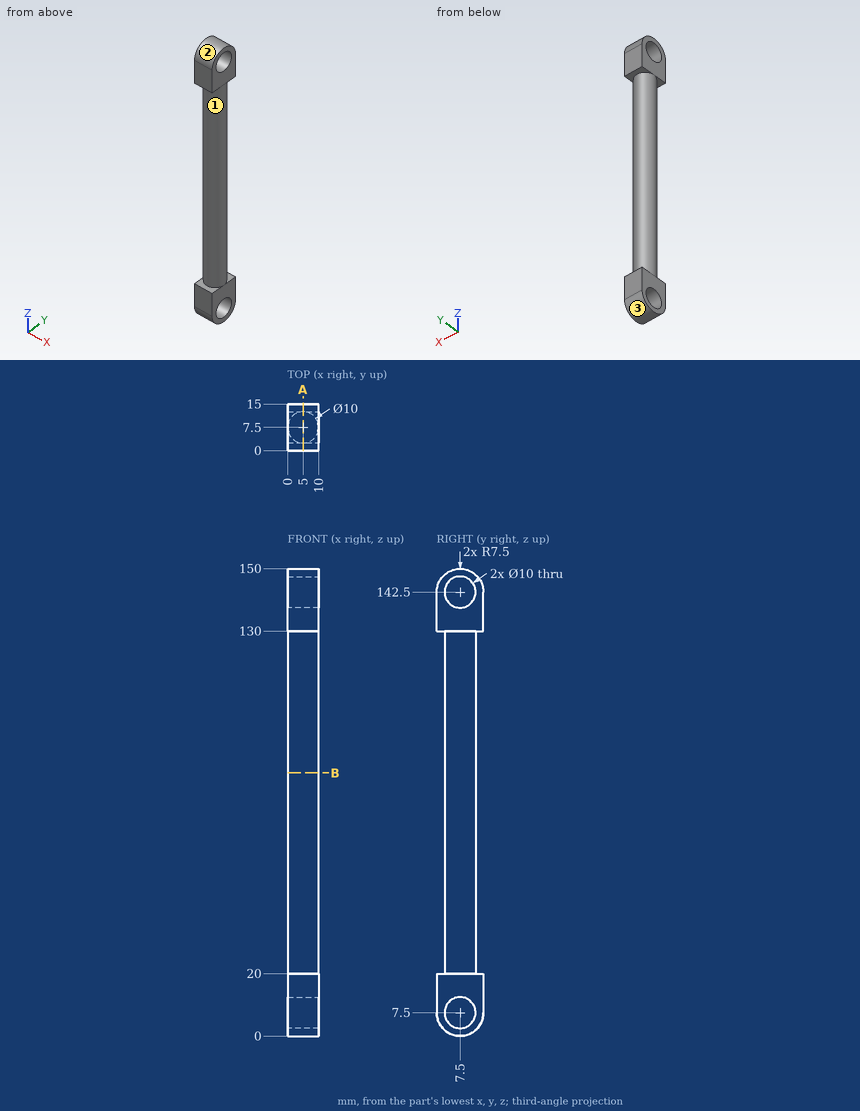
Design review of the part shown in the three views and the two pictorial views. Dimensions are in mm from the part's minimum x, y and z. Coordinates: 2 decimals unless noted, no trailing zeros. Order: outer loops, then holes, each group sorted by start corner. A loop starts at its lowest first (then second) coordinate and runs counter-clockwise, first axis right, second up. Notation, with made-up numbers: (53, 53.5) - (98, 53.5) arc R25 cw to (98, 66.5) - close; hole circle Ø6 at (60.25, 12). An arc over 180 degrees is marked (long way). Answer as CSV lines item,"result". Start each with the question number.
1) Draft analysis for pull direction Z (two halves, no side actions). For the marked faces 1, 2 and 3, state which applies: +Z half, -Z half, draft (parallel to the pull), parting line (faces both ways), or undercut.
2) Add section A-A (x = 5). State the section outline as (y, z) points, then the cut area to 3 significant figures.
3) Insertion check: P1, Ø3, axis at x = 8.5, z = 52.5, coming from the +Y side; P2, Ø2.5, axis at x = 3.5, y = 3.5, coming from the +Z side; P3, Ø3.5, axis at x = 4.5, y = 13, coming from the +Z side; P4, Ø6, axis at x = 4, y = 4.5, coming from the -Z side. Each pin has a flat end and moves straight along its axis. Give the tip position at first contact, or say it passes through.
4) To check wall thickness, follow line 1 along Z through (x, y) = (1.5, 7); line 2 along Y through (x, z) = (4.5, 7.5); line 3 along Z through (x, y) = (9.25, 9.5). State the ranges of each line that lie inside material, in increasing order. Write a range as [from, to].
5) Add section B-B (z = 84.5). State the section outline as (x, y) points, then the cut area to 3 significant figures.
Result:
1,face 1,"undercut"
1,face 2,"+Z half"
1,face 3,"-Z half"
2,outline,"(0, 7.5) arc R7.5 ccw to (15, 7.5) - (15, 20) - (12.5, 20) - (12.5, 130) - (15, 130) - (15, 142.5) arc R7.5 ccw to (0, 142.5) - (0, 130) - (2.5, 130) - (2.5, 20) - (0, 20) - close; hole circle Ø10 at (7.5, 7.5); hole circle Ø10 at (7.5, 142.5)"
2,area,"1,490 mm^2"
3,P1,"y = 12.08"
3,P2,"z = 149.48"
3,P3,"z = 149"
3,P4,"z = 0"
4,line 1,"[0.02, 2.53], [12.47, 137.53], [147.47, 149.98]"
4,line 2,"[0, 2.5], [12.5, 15]"
4,line 3,"[0.27, 2.92], [12.08, 137.92], [147.08, 149.73]"
5,outline,"circle Ø10 at (5, 7.5)"
5,area,"78.5 mm^2"
